Here's how the part is built. I have some questions about the finished solid (model axes, mm). Face numbers are marked on the shaded views. A direction names the side the tool comes from. Give positions to 0.01 mm unless a question says otherwise; leave off trailing zeros. Loops run counter-clockwise (first coordinate to the right, second up) from the corner with the lowest first, then second, coordinate; pieces in that order, holes last.
Q1. I need wall thicknesses on probe 1 along Y at (x, z) = (-5.5, 40); probe 2 along Y at (x, z) = (56.5, 18); probe 3 along Z at (x, y) = (27, 47). Which ranges of each line are inside material? Lowest first, please.
Q2. I'm going to push flat-ended pins straight in: P1, Ø10, axis at y = 81, z = 158, coming from the +X side; P2, Ø6, axis at y = 42, z = 82, coming from the -X side; P3, Ø12, axis at x = -4, z = 124, coming from the +Y side; P4, Ø16.5, axis at x = -7, z = 109, coming from the -Y side. Where does each tip first touch, or does it pass through?
Q3. Suppose I cut it at C-C (x = 54.5). List the corners of the cut face in (y, z) for me.
Q4. Suppose I cut it at B-B (z = 40). List the corners of the cut face in (x, y) for me, and give its area (3 significant figures).
Q5. Thinking about a two-plate mould opening in Y: for the marked faces 1, 2 and 3, which applies, pulls with the +Y half, pulls with the -Y half, needs draft (parallel to the pull), parting line crosses it, or undercut?
Q6. For the marked faces 4, 5, 6, 7 and 8, which set-ups out of +Z, -Z, +X, -X, +Y, -Y let a thin tool reach every point of the face, with its end or its side?
Q7. Suppose I cut it at D-D (x = -5). List the corners of the cut face in (y, z) for me, and give its area (3 significant figures).
Q8. Suppose I cut it at A-A (y = 50). List the corners of the cut face in (x, z) for me.
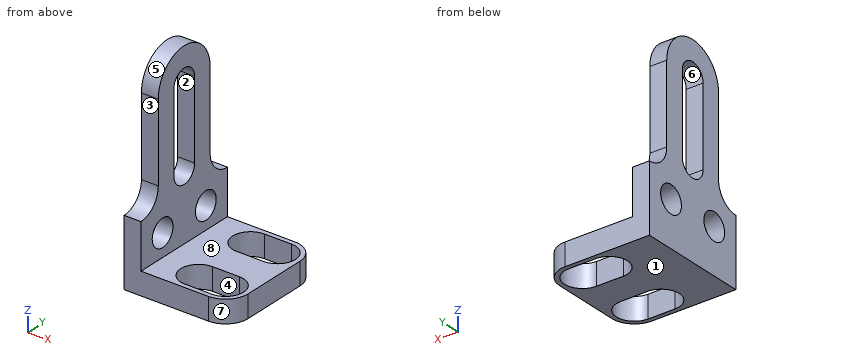
```python
from build123d import *

# Parameters (mm, degrees)
BASE_BLOCK_DEPTH    = 20
UPRIGHT_PLATE_DEPTH = 15
SLOTTED_ARM_DEPTH   = 15
HOLES_2X_SKETCH_R   = 12
HOLES_2X_DEPTH      = 15
SLOTS_2X_DEPTH      = 20


with BuildPart() as part:
    # Base Block Sketch → Base Block (new body)
    with BuildSketch(Plane.XY):
        with BuildLine():
            Line((0, 0), (60, 0))
            ThreePointArc((60, 0), (74.142135624, 5.857864376), (80, 20))
            Line((80, 20), (80, 80))
            ThreePointArc((80, 80), (74.142135624, 94.142135624), (60, 100))
            Line((60, 100), (0, 100))
            Line((0, 100), (0, 0))
        make_face()
    extrude(amount=BASE_BLOCK_DEPTH)

    # Upright Plate Sketch → Upright Plate (add)
    with BuildSketch(Plane.ZY):
        Polygon((20, 0), (60, 0), (60, 100), (0, 100), (0, 0), align=None)
    extrude(amount=UPRIGHT_PLATE_DEPTH)

    # Slotted Arm Sketch → Slotted Arm (add)
    with BuildSketch(Plane.ZY.offset(15)):
        with BuildLine():
            Line((150, 80), (80, 80))
            ThreePointArc((80, 80), (65.857864376, 85.857864376), (60, 100))
            Line((60, 100), (60, 0))
            ThreePointArc((60, 0), (65.857864376, 14.142135624), (80, 20))
            Line((80, 20), (150, 20))
            ThreePointArc((150, 20), (180, 50), (150, 80))
        make_face()
        with BuildLine():
            Line((80, 62), (150, 62))
            ThreePointArc((150, 62), (162, 50), (150, 38))
            Line((150, 38), (80, 38))
            ThreePointArc((80, 38), (68, 50), (80, 62))
        make_face(mode=Mode.SUBTRACT)
    extrude(amount=-SLOTTED_ARM_DEPTH)

    # Holes 2x Sketch → Holes 2x (cut)
    with BuildSketch(Plane(origin=(0, 0, 0), x_dir=(0, 0, -1), z_dir=(1, 0, 0))):
        with Locations((-40, 75)):
            Circle(HOLES_2X_SKETCH_R)
        with Locations((-40, 25)):
            Circle(HOLES_2X_SKETCH_R)
    extrude(amount=-HOLES_2X_DEPTH, mode=Mode.SUBTRACT)

    # Slots 2x Sketch → Slots 2x (cut)
    with BuildSketch(Plane.XY.offset(20)):
        with BuildLine():
            Line((36, 96), (60, 96))
            ThreePointArc((60, 96), (76, 80), (60, 64))
            Line((60, 64), (36, 64))
            ThreePointArc((36, 64), (20, 80), (36, 96))
        make_face()
        with BuildLine():
            Line((36, 36), (60, 36))
            ThreePointArc((60, 36), (76, 20), (60, 4))
            Line((60, 4), (36, 4))
            ThreePointArc((36, 4), (20, 20), (36, 36))
        make_face()
    extrude(amount=-SLOTS_2X_DEPTH, mode=Mode.SUBTRACT)


solid = part.part
```
Solutions:
1. probe 1: y = 0 to 13, 37 to 63, 87 to 100
1. probe 2: y = 0 to 4, 36 to 64, 96 to 100
1. probe 3: z = 0 to 20
2. P1: stops at x = 0
2. P2: passes through
2. P3: stops at y = 80
2. P4: stops at y = 20
3. outline: (0, 0) - (4, 0) - (4, 20) - (0, 20) - close; (36, 0) - (64, 0) - (64, 20) - (36, 20) - close; (96, 0) - (100, 0) - (100, 20) - (96, 20) - close
4. outline: (-15, 0) - (0, 0) - (0, 13) - (-15, 13) - close; (-15, 37) - (0, 37) - (0, 63) - (-15, 63) - close; (-15, 87) - (0, 87) - (0, 100) - (-15, 100) - close
4. area: 780 mm2
5. face 1: needs draft
5. face 2: undercut
5. face 3: pulls with the -Y half
6. face 4: +Z, -Z
6. face 5: +Z, +X, -X
6. face 6: +X, -X
6. face 7: +Z, -Z, +X, -Y
6. face 8: +Z, +X, +Y, -Y
7. outline: (0, 0) - (100, 0) - (100, 60) arc R20 cw to (80, 80) - (80, 150) arc R30 ccw to (20, 150) - (20, 80) arc R20 cw to (0, 60) - close; hole circle Ø24 at (25, 40); hole (38, 80) arc R12 ccw to (62, 80) - (62, 150) arc R12 ccw to (38, 150) - close; hole circle Ø24 at (75, 40)
7. area: 9,950 mm2
8. outline: (-15, 0) - (80, 0) - (80, 20) - (0, 20) - (0, 68) - (-15, 68) - close; (-15, 162) - (0, 162) - (0, 180) - (-15, 180) - close
